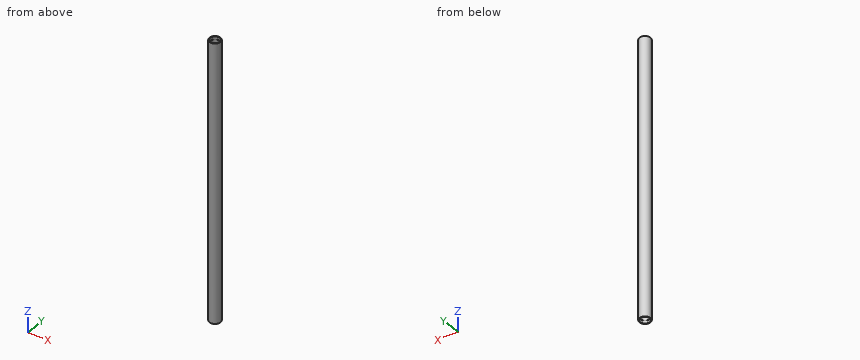
```python
from build123d import *

# Parameters (mm, degrees)
SKETCH_1_R          = 30
EXTRUDE_1_DEPTH     = 1480
SKETCH_2_R          = 24
CUT_EXTRUDE_1_DEPTH = 1600
SKETCH_3_R          = 26
CUT_EXTRUDE_2_DEPTH = 15
CUT_EXTRUDE_START   = -15
SKETCH_4_R          = 26
CUT_EXTRUDE_3_DEPTH = 15
CHAMFER_1_SIZE      = 0.5


with BuildPart() as part:
    # 草图1 → 凸台-拉伸1 (new body)
    with BuildSketch(Plane.XY):
        Circle(SKETCH_1_R)
    extrude(amount=EXTRUDE_1_DEPTH)

    # 草图2 → 切除-拉伸1 (cut)
    with BuildSketch(Plane(origin=(0, 0, 0), x_dir=(-1, 0, 0), z_dir=(0, 0, -1))):
        Circle(SKETCH_2_R)
    extrude(amount=-CUT_EXTRUDE_1_DEPTH, mode=Mode.SUBTRACT)

    # 草图3 → 切除-拉伸2 (cut)
    with BuildSketch(Plane(origin=(0, 0, 0), x_dir=(-1, 0, 0), z_dir=(0, 0, -1))):
        Circle(SKETCH_3_R)
    extrude(amount=-CUT_EXTRUDE_2_DEPTH, mode=Mode.SUBTRACT)

    # 草图4 → 切除-拉伸3 (cut)
    with BuildSketch(Plane.XY.offset(1480).offset(CUT_EXTRUDE_START)):
        with Locations(Location((0, 0, 0), (0, 0, 180))):
            Circle(SKETCH_4_R)
    extrude(amount=CUT_EXTRUDE_3_DEPTH, mode=Mode.SUBTRACT)

    # 倒角1
    chamfer_1_edges = [part.edges().sort_by_distance(p)[0] for p in [
        (26, 0, 0),
        (-30, 0, 0),
        (26, 0, 1480),
        (-30, 0, 1480),
    ]]
    chamfer(chamfer_1_edges, length=CHAMFER_1_SIZE)


solid = part.part
```
Input: part model. Units: mm. Frame: model coordinates. Round coordinates to 2 decimals unless told otherwise and drop trailing zeros. Loops run counter-clockwise (first coordinate to the right, second up) from the corner with the lowest first, then second, coordinate; pieces in that order, holes last. Notation, with made-up numbers: (25, 72) -> (42, 72) arc R17 ccw to (42, 100) -> close; hole circle Ø4 at (-12, 73). An arc over 180 degrees is marked (long way). Use one line per item in the form item = value. Start each with the question number.
Item 1: Section query C-C on z = 178.5. Return the cut outline in (x, y), then the cut area to 3 significant figures.
Item 2: Material intervals for L1, parallel to Y at x = -3, z = 1134; L2, parallel to Y at x = 0, z = 619; L3, parallel to X at y = -20, z = 1221.5, sorted ascending. Write a range as from..to.
Item 3: Section query A-A on y = 0. Return the cut outline in (x, z), then the cut area to 3 significant figures.
Item 4: Contact query for flat-ended pins moving along their axis: pin 1 Ø8 at (x, z) = (22.5, 387.5) entering from +Y; pin 2 Ø4 at (x, z) = (-9, 1097.5) entering from -Y; pin 3 Ø5 at (x, z) = (15.5, 865.5) entering from -Y. Output: stop coordinate, or through.
Ans:
q1.outline = circle Ø60 at (0, 0); hole circle Ø48 at (0, 0)
q1.area = 1,020 mm^2
q2.L1 = -29.85..-23.81, 23.81..29.85
q2.L2 = -30..-24, 24..30
q2.L3 = -22.36..-13.27, 13.27..22.36
q3.outline = (-30, 0.5) -> (-29.5, 0) -> (-26.5, 0) -> (-26, 0.5) -> (-26, 15) -> (-24, 15) -> (-24, 1465) -> (-26, 1465) -> (-26, 1479.5) -> (-26.5, 1480) -> (-29.5, 1480) -> (-30, 1479.5) -> close; (24, 15) -> (26, 15) -> (26, 0.5) -> (26.5, 0) -> (29.5, 0) -> (30, 0.5) -> (30, 1479.5) -> (29.5, 1480) -> (26.5, 1480) -> (26, 1479.5) -> (26, 1465) -> (24, 1465) -> close
q3.area = 17,600 mm^2
q4.pin_1 = 23.62
q4.pin_2 = -29.17
q4.pin_3 = -27.04
